The listing builds one solid part. Answer for the finished solid, in the listing's coordinates (mm). Face numbers are marked on the shaded views. A direction names the side the tool comes from. Coordinates: 2 decimals unless noted, no trailing zeros. Order: outer loops, then holes, each group sorted by start corner. A loop starts at its lowest first (then second) coordinate and runs counter-clockwise, first axis right, second up.
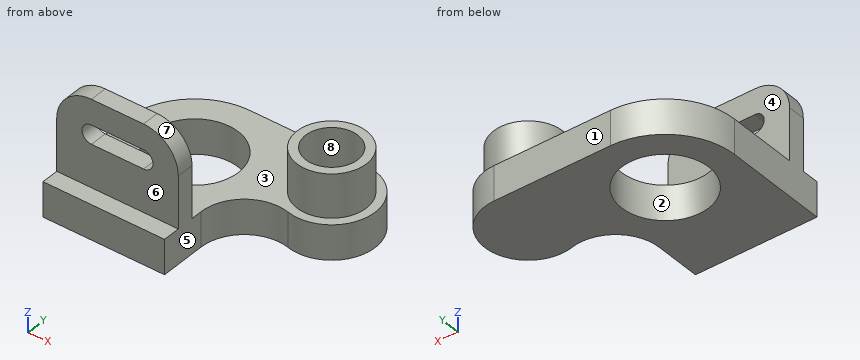
from build123d import *

# Parameters (mm, degrees)
UPRIGHT_PLATE_DEPTH             = 20
BEARING_BOSS_PROFILE_R          = 20
BEARING_BOSS_PROFILE_R_2        = 15
BEARING_BOSS_DEPTH              = 25
BEARING_BORE_SKETCH_R           = 25
BEARING_BORE_50_DEPTH           = 168.478356811
BASE_PLATE_PROFILE_W            = 70
BASE_PLATE_PROFILE_H            = 10
BASE_PLATE_DEPTH                = 50
BASE_PLATE_CORNER_FILLETS_R20_R = 20
MOUNTING_SLOT_DEPTH             = 170.481562419


with BuildPart() as part:
    # Upright Plate Profile → Upright Plate (new body)
    with BuildSketch(Plane.XY):
        with BuildLine():
            Line((0, 0), (70, 0))
            Line((70, 0), (70, 26.461355602))
            ThreePointArc((70, 26.461355602), (79.588964993, 46.146375287), (101, 50.730677801))
            ThreePointArc((101, 50.730677801), (131.816658266, 71.977836452), (107, 100))
            Line((107, 100), (40, 100))
            ThreePointArc((40, 100), (11.715728753, 88.284271247), (0, 60))
            Line((0, 60), (0, 0))
        make_face()
    extrude(amount=UPRIGHT_PLATE_DEPTH)

    # Bearing Boss Profile → Bearing Boss (add)
    with BuildSketch(Plane.XY.offset(20)):
        with Locations(Location((107, 75, 0), (0, 0, 180))):
            Circle(BEARING_BOSS_PROFILE_R)
        with Locations((107, 75)):
            Circle(BEARING_BOSS_PROFILE_R_2, mode=Mode.SUBTRACT)
    extrude(amount=BEARING_BOSS_DEPTH)

    # Bearing Bore Sketch → Bearing Bore Ø50 (cut, through all)
    with BuildSketch(Plane.XY.offset(20)):
        with Locations((40, 60)):
            Circle(BEARING_BORE_SKETCH_R)
    extrude(amount=-BEARING_BORE_50_DEPTH, mode=Mode.SUBTRACT)

    # Base Plate Profile → Base Plate (add)
    with BuildSketch(Plane.XY.offset(20)):
        with Locations((35, 15)):
            Rectangle(BASE_PLATE_PROFILE_W, BASE_PLATE_PROFILE_H)
    extrude(amount=BASE_PLATE_DEPTH)

    # Base Plate Corner Fillets R20
    base_plate_corner_fillets_r20_edges = [part.edges().sort_by_distance(p)[0] for p in [
        (70, 15, 70),
        (0, 15, 70),
    ]]
    fillet(base_plate_corner_fillets_r20_edges, radius=BASE_PLATE_CORNER_FILLETS_R20_R)

    # Mounting Slot Sketch → Mounting Slot (cut, through all)
    with BuildSketch(Plane(origin=(0, 20, 0), x_dir=(1, 0, 0), z_dir=(0, 1, 0))):
        with BuildLine():
            Line((20, -44.564709442), (50, -44.564709442))
            ThreePointArc((50, -44.564709442), (55.435290558, -50), (50, -55.435290558))
            Line((50, -55.435290558), (20, -55.435290558))
            ThreePointArc((20, -55.435290558), (14.564709442, -50), (20, -44.564709442))
        make_face()
    extrude(amount=-MOUNTING_SLOT_DEPTH, mode=Mode.SUBTRACT)


solid = part.part
1) A tool of negligible diameter and unlimited length cuts with its end or side. For the marked faces 4, 5, 6, 7 and 8, from which of +Z, -Z, +X, -X, +Y, -Y can it reach the whole face along a straight path? Write none if from no direction.
2) Consider L1, parallel to Y at x = 40, z = 10.25; L2, parallel to Z at x = 22, y = 16.5; L3, parallel to Y at x = 65.5, z = 44. Determine where each line is inside the solid, lowest interval first.
3) Section D-D (z = 9.5) is taken. Give the vertices of the cut face in (x, y).
4) Determine the mould class of the marked faces 1, 2 and 3 for opening direction Y: released by +Y, released by -Y, zero draft, split by the parting line, or undercut.
5) Section A-A (z = 31.5) is taken. Give the vertices of the cut face in (x, y), then the cut area to 3 significant figures.
6) Section B-B (y = 75) is taken. Give the vertices of the cut face in (x, z).
7) Section C-C (x = 94.5) is taken. Give the vertices of the cut face in (y, z).
8) Each of these flat-tipped pins is pushed along its axis until it touches: P1, Ø1, axis at x = 15.5, z = 40.5, coming from the +Y side; P2, Ø3, axis at x = 50, y = 5, coming from the +Z side; P3, Ø21, axis at y = 19, z = 18.5, coming from the +X side. Where does it stop, or does it pass through?
Filled sheet:
1. face 4: +Z, +X, -X, +Y
1. face 5: +Z, -Z, +X, -Y
1. face 6: +Z, +X, -X, -Y
1. face 7: +Z, +X, +Y, -Y
1. face 8: +Z
2. L1: y = 0 to 35, 85 to 100
2. L2: z = 0 to 44.56, 55.44 to 70
2. L3: y = 10 to 20
3. outline: (0, 0) - (70, 0) - (70, 26.46) arc R25 cw to (101, 50.73) arc R25 ccw (long way) to (107, 100) - (40, 100) arc R40 ccw to (0, 60) - close; hole circle Ø50 at (40, 60)
4. face 1: released by +Y
4. face 2: undercut
4. face 3: zero draft
5. outline: (0, 10) - (70, 10) - (70, 20) - (0, 20) - close; circle Ø40 at (107, 75); hole circle Ø30 at (107, 75)
5. area: 1,250 mm2
6. outline: (2.92, 0) - (20, 0) - (20, 20) - (2.92, 20) - close; (60, 0) - (132, 0) - (132, 20) - (127, 20) - (127, 45) - (122, 45) - (122, 20) - (92, 20) - (92, 45) - (87, 45) - (87, 20) - (60, 20) - close
7. outline: (51.46, 0) - (100, 0) - (100, 20) - (90.61, 20) - (90.61, 45) - (83.29, 45) - (83.29, 20) - (66.71, 20) - (66.71, 45) - (59.39, 45) - (59.39, 20) - (51.46, 20) - close
8. P1: stops at y = 20
8. P2: stops at z = 20
8. P3: stops at x = 70.19
